```python
from build123d import *

# Parameters (mm, degrees)
SKETCH1_R             = 1.5
BOSS_EXTRUDE1_DEPTH   = 3
M4_TAPPED_HOLE1_D     = 3.3
M4_TAPPED_HOLE1_DEPTH = 11.5
M4_TAPPED_HOLE1_TIP   = 0.991420021
CHAMFER1_SIZE         = 0.5
CHAMFER2_SIZE         = 0.5
CHAMFER3_SIZE         = 0.5


with BuildPart() as part:
    # Sketch1 → Boss-Extrude1 (new body)
    with BuildSketch(Plane.XY):
        with BuildLine():
            Line((-2.8, 3.8), (2.8, 3.8))
            ThreePointArc((2.8, 3.8), (3.507106781, 3.507106781), (3.8, 2.8))
            Line((3.8, 2.8), (3.8, -2.8))
            ThreePointArc((3.8, -2.8), (3.507106781, -3.507106781), (2.8, -3.8))
            Line((2.8, -3.8), (-2.8, -3.8))
            ThreePointArc((-2.8, -3.8), (-3.507106781, -3.507106781), (-3.8, -2.8))
            Line((-3.8, -2.8), (-3.8, 2.8))
            ThreePointArc((-3.8, 2.8), (-3.507106781, 3.507106781), (-2.8, 3.8))
        make_face()
        Circle(SKETCH1_R, mode=Mode.SUBTRACT)
    extrude(amount=BOSS_EXTRUDE1_DEPTH)

    # M4 Tapped Hole1
    with Locations(Plane(origin=(0, 0, 0), x_dir=(-1, 0, 0), z_dir=(0, 0, -1))):
        with Locations((0, 0)):
            Hole(M4_TAPPED_HOLE1_D / 2, depth=M4_TAPPED_HOLE1_DEPTH)
            with Locations((0, 0, -(M4_TAPPED_HOLE1_DEPTH + M4_TAPPED_HOLE1_TIP / 2))):  # 118° drill point
                Cone(0, M4_TAPPED_HOLE1_D / 2, M4_TAPPED_HOLE1_TIP, mode=Mode.SUBTRACT)

    # Chamfer1
    chamfer1_edges = [part.edges().sort_by_distance(p)[0] for p in [
        (-1.65, 0, 0),
    ]]
    chamfer(chamfer1_edges, length=CHAMFER1_SIZE)

    # Chamfer2
    chamfer2_edges = [part.edges().sort_by_distance(p)[0] for p in [
        (-1.65, 0, 3),
    ]]
    chamfer(chamfer2_edges, length=CHAMFER2_SIZE)

    # Chamfer3
    chamfer3_edges = [part.edges().sort_by_distance(p)[0] for p in [
        (3.507106781, -3.507106781, 3),
        (0, -3.8, 0),
        (-3.507106781, -3.507106781, 0),
        (3.8, 0, 3),
        (3.507106781, 3.507106781, 3),
        (0, 3.8, 3),
        (-3.507106781, 3.507106781, 3),
        (-3.8, 0, 3),
        (-3.507106781, -3.507106781, 3),
        (0, -3.8, 3),
        (-3.8, 0, 0),
        (-3.507106781, 3.507106781, 0),
        (0, 3.8, 0),
        (3.507106781, 3.507106781, 0),
        (3.8, 0, 0),
        (3.507106781, -3.507106781, 0),
    ]]
    chamfer(chamfer3_edges, length=CHAMFER3_SIZE)


solid = part.part
```
For this review, take the finished solid that the model builds, in its own axes (mm). Give positions to 0.01 mm unless a question says otherwise; leave off trailing zeros. Loops run counter-clockwise (first coordinate to the right, second up) from the corner with the lowest first, then second, coordinate; pieces in that order, holes last. Notation, with made-up numbers: M 16,48 L 53,48 A15 cw 53,69 Z; hole C 67,21 d8. An arc over 180 degrees is marked long. One line per item, written item: value. Start each with the question number.
Q1. For L1, parallel to Y at x = 0, z = 1.2; L2, parallel to X at y = -1, z = 1.6; L3, parallel to X at y = 1.25, z = 0.75, list the stretches that pass through material, from the lowest coordinate up.
Q2. Clearance check with a flat-ended pin moving along its axis: pin 1 Ø2.5 at (x, y) = (0, 0) entering from -Z. State where the tip first meets the part, or that it passes through.
Q3. Draft analysis for pull direction Y (two halves, no side actions). For faces 1 (the face through (-3.515, 3.499, 1.486)), 2 (the face through (-0.7, 2.2, 3)), 3 (the face through (-1.216, 1.115, 1.514)), state which applies: released by +Y, released by -Y, zero draft, split by the parting line, or undercut.
Q4. Add section A-A (x = 0). Give the boundary of the cut face in (y, z), and give its area (3 significant figures).
Q5. Add section D-D (y = -2.25). Give the boundary of the cut face in (x, z).
Q6. Add section B-B (z = 2.7). Give the boundary of the cut face in (x, y), and give its area (3 significant figures).
Reply:
1. L1: -3.8 to -1.65, 1.65 to 3.8
1. L2: -3.8 to -1.31, 1.31 to 3.8
1. L3: -3.8 to -1.08, 1.08 to 3.8
2. pin 1: through
3. face 1: released by +Y
3. face 2: zero draft
3. face 3: undercut
4. outline: M -3.8,0.5 L -3.3,0 L -2.15,0 L -1.65,0.5 L -1.65,2.5 L -2.15,3 L -3.3,3 L -3.8,2.5 Z; M 1.65,0.5 L 2.15,0 L 3.3,0 L 3.8,0.5 L 3.8,2.5 L 3.3,3 L 2.15,3 L 1.65,2.5 Z
4. area: 11.9 mm²
5. outline: M -3.8,0.5 L -3.3,0 L 3.3,0 L 3.8,0.5 L 3.8,2.5 L 3.3,3 L -3.3,3 L -3.8,2.5 Z
6. outline: M -3.6,-2.8 A0.8 ccw -2.8,-3.6 L 2.8,-3.6 A0.8 ccw 3.6,-2.8 L 3.6,2.8 A0.8 ccw 2.8,3.6 L -2.8,3.6 A0.8 ccw -3.6,2.8 Z; hole C 0,0 d3.7
6. area: 40.5 mm²
